Check sheet for the drawn part. Datum: minimum x, y, z corner. Units: mm. Give positions to 0.01 mm unless a question says otherwise; leave off trailing zeros. Write each loop counter-clockwise with the first axis right and the second up, starting at its lowest first coordinate (ties: lowest second). Pieces come first, ordered by that corner, then holes.
(1) Cross-section at A-A (z = 19.75). Record the boundary of the cut face in (x, y), and give its area (3 significant figures).
(2) Depth check by flat-ended pin: P1, Ø9, axis at x = 22, z = 21.5, coming from the +Y side; P2, Ø15, axis at y = 777, z = 14, coming from the -X side. Enter the tip coordinate at first touch or a pass-through.
(3) Thickness scan on line 1 along X through (y, z) = (731, 12); line 2 along Y through (x, z) = (42.5, 4.5); line 3 along X through (y, z) = (691.5, 27). Record the ranges inside material, lowest first.
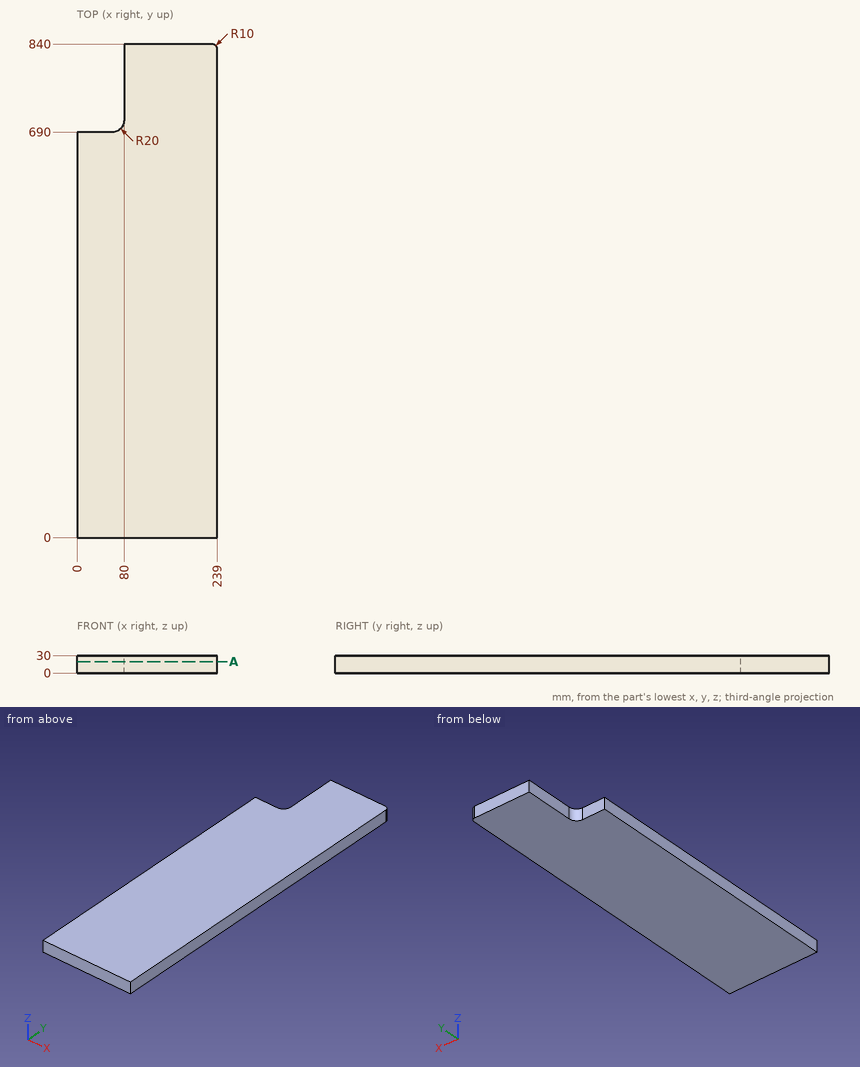
Reply:
1. outline: (0, 0) - (239, 0) - (239, 830) arc R10 ccw to (229, 840) - (80, 840) - (80, 710) arc R20 cw to (60, 690) - (0, 690) - close
1. area: 189,000 mm2
2. P1: stops at y = 690
2. P2: stops at x = 80
3. line 1: x = 80 to 239
3. line 2: y = 0 to 690
3. line 3: x = 67.6 to 239
